Verification items for this drawing (mm, ordinates from the low corner). A direction names the side the tool comes from. Give positions to 0.01 mm unless a question says otherwise; leave off trailing zeros. Order: outer loops, then holes, each group sorted by start corner. A loop starts at its lowest first (then second) coordinate and runs counter-clockwise, first axis right, second up. Notation, with made-up numbers: M 57,79 L 106,79 A26 cw 106,116 Z; hole C 46.5,-6.75 d4. An arc over 180 degrees is marked long. Return JSON: item names as keys, results as strings. Group by question number.
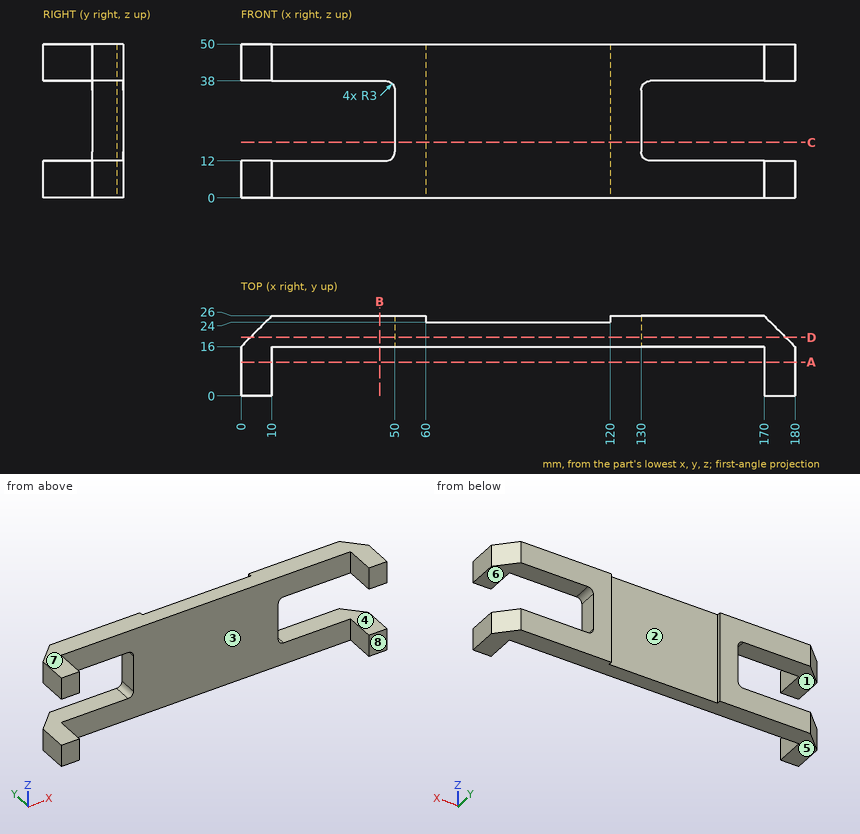
1) Depth check by flat-ended pin: P1, Ø2, axis at y = 18, z = 11, coming from the -X side; P2, Ø15, axis at x = 83, z = 31.5, coming from the +Y side; P3, Ø10, axis at x = 107.5, y = 9, coming from the -Z side; P4, Ø5, axis at y = 21, z = 27.5, coming from the +X side. Enter the tip coordinate at first touch or a pass-through.
2) Sectioned sample at A-A on y = 11. Record the boundary of the cut face in (x, z), then the cut area to 3 significant figures.
3) Sectioned sample at C-C on z = 18. Record the boundary of the cut face in (x, y).
4) Sectioned sample at B-B on x = 45. Record the boundary of the cut face in (y, z).
5) Release check for a two-part mould opening along Z. For the marked faces 5, 6, 7 and 8 record: released by +Z, released by -Z, zero draft, split by the parting line, or undercut.
6) Material ranges on line 1 along Z through (x, y) = (26, 21); line 2 along X through (y, z) = (24.5, 31.5); line 3 along X through (y, z) = (12, 45), recorded low to high.
7) Tool access check on the marked faces 1, 2, 3 and 4. Record the directions out of +Z, -Z, +X, -X, +Y, -Y that give a thin tool (end or side, any length) a straight path to the whole face; none if there is none.
8) Sectioned sample at D-D on y = 19. Record the boundary of the cut face in (x, z), then the cut area to 3 significant figures.
Reply:
{
 "1": {"P1": "x = 1", "P2": "y = 24", "P3": "through", "P4": "x = 130"},
 "2": {"outline": "M 0,0 L 10,0 L 10,12 L 0,12 Z; M 0,38 L 10,38 L 10,50 L 0,50 Z; M 170,0 L 180,0 L 180,12 L 170,12 Z; M 170,38 L 180,38 L 180,50 L 170,50 Z", "area": "480 mm^2"},
 "3": {"outline": "M 50,16 L 130,16 L 130,26 L 120,26 L 120,24 L 60,24 L 60,26 L 50,26 Z"},
 "4": {"outline": "M 16,0 L 26,0 L 26,12 L 16,12 Z; M 16,38 L 26,38 L 26,50 L 16,50 Z"},
 "5": {"face 5": "released by -Z", "face 6": "undercut", "face 7": "released by +Z", "face 8": "zero draft"},
 "6": {"line 1": "0 to 12, 38 to 50", "line 2": "50 to 60, 120 to 130", "line 3": "0 to 10, 170 to 180"},
 "7": {"face 1": "-X, +Y, -Y", "face 2": "+Z, -Z, +Y", "face 3": "+Z, -Z, -Y", "face 4": "+X, +Y, -Y"},
 "8": {"outline": "M 3,0 L 177,0 L 177,12 L 133,12 A3 cw 130,15 L 130,35 A3 cw 133,38 L 177,38 L 177,50 L 3,50 L 3,38 L 47,38 A3 cw 50,35 L 50,15 A3 cw 47,12 L 3,12 Z", "area": "6,260 mm^2"}
}
